Verification items for the finished model (mm, model axes). A direction names the side the tool comes from. Coordinates: 2 decimals unless noted, no trailing zeros. Write each loop counter-clockwise with the first axis right and the second up, starting at its lowest first coordinate (ties: lowest second). Pieces come first, ordered by that corner, then holes. Notation, with made-up numbers: (25, 7) -> (38, 7) arc R23 cw to (38, 41) -> close; hole circle Ø10 at (26.25, 33.25). An arc over 180 degrees is marked (long way). Answer in a Markdown table with one row per item.
```python
from build123d import *

# Parameters (mm, degrees)
EXTRUDE_1_DEPTH         = 115
SKETCH_2_W              = 200
SKETCH_2_H              = 37
EXTRUDE_2_DEPTH         = 30
EXTRUDE_3_DEPTH         = 20
SKETCH_4_R              = 22.5
CUT_EXTRUDE_1_DEPTH     = 2
SKETCH_5_R              = 18.5
CUT_EXTRUDE_2_DEPTH     = 8
CUT_EXTRUDE_3_REACH     = 169.29
SKETCH_6_R              = 23.5
SKETCH_7_R              = 9.5
CUT_EXTRUDE_4_DEPTH     = 85
SKETCH_8_R              = 6.5
CUT_EXTRUDE_5_DEPTH     = 154.186161255
SKETCH_9_R              = 2.5
CUT_EXTRUDE_6_DEPTH     = 10
FILLET_1_R              = 5
SKETCH_10_R             = 1
CUT_EXTRUDE_7_DEPTH     = 5
M5X0_8_1_D              = 4.2
M5X0_8_1_DEPTH          = 11
M5X0_8_1_TIP            = 1.2618073
HOLE_WIZARD_M10_1_D     = 8.5
HOLE_WIZARD_M10_1_DEPTH = 24
HOLE_WIZARD_M10_1_TIP   = 2.553657631
SKETCH_15_R             = 6.5
CUT_EXTRUDE_8_DEPTH     = 55
SKETCH_16_R             = 9.5
CUT_EXTRUDE_9_DEPTH     = 12


with BuildPart() as part:
    # 草图1 → 拉伸1 (new body)
    with BuildSketch(Plane.XY):
        Polygon((80, 0), (-80, 0), (-100, -20), (-100, -42), (100, -42), (100, -20), align=None)
    extrude(amount=EXTRUDE_1_DEPTH)

    # 草图2 → 拉伸2 (add)
    with BuildSketch(Plane.XY):
        with Locations((0, -60.5)):
            Rectangle(SKETCH_2_W, SKETCH_2_H)
    extrude(amount=EXTRUDE_2_DEPTH)

    # 草图3 → 拉伸3 (add)
    with BuildSketch(Plane.ZY.offset(100)):
        Polygon((115, -42), (30, -79), (30, -42), align=None)
    extrude_3 = extrude(amount=-EXTRUDE_3_DEPTH)

    # 镜向1: 拉伸3 across plane
    add(extrude_3.mirror(Plane(origin=(0, 0, 0), x_dir=(0, 0, 1), z_dir=(1, 0, 0))))

    # 草图4 → 切除-拉伸1 (cut)
    with BuildSketch(Plane(origin=(0, 0, 0), x_dir=(1, 0, 0), z_dir=(0, 1, 0))):
        with Locations(Location((0, -70, 0), (0, 0, 270))):
            Circle(SKETCH_4_R)
    extrude(amount=-CUT_EXTRUDE_1_DEPTH, mode=Mode.SUBTRACT)

    # 草图5 → 切除-拉伸2 (cut)
    with BuildSketch(Plane(origin=(0, -2, 0), x_dir=(1, 0, 0), z_dir=(0, 1, 0))):
        with Locations(Location((0, -70, 0), (0, 0, 270))):
            Circle(SKETCH_5_R)
    extrude(amount=-CUT_EXTRUDE_2_DEPTH, mode=Mode.SUBTRACT)

    # 草图6 → 切除-拉伸3 (cut, up to next)
    with BuildSketch(Plane(origin=(0, -10, 0), x_dir=(1, 0, 0), z_dir=(0, 1, 0)), mode=Mode.PRIVATE) as cut_extrude_3_sk1:
        with Locations(Location((0, -70, 0), (0, 0, 270))):
            Circle(SKETCH_6_R)
    cut_extrude_3_tool1 = extrude(cut_extrude_3_sk1.sketch, amount=-CUT_EXTRUDE_3_REACH, mode=Mode.PRIVATE) & part.part
    add(cut_extrude_3_tool1.solids().sort_by_distance((0, -10, 70))[0], mode=Mode.SUBTRACT)

    # 草图7 → 切除-拉伸4 (cut)
    with BuildSketch(Plane.XY.offset(115)):
        with Locations((60, -21)):
            Circle(SKETCH_7_R)
        with Locations((-60, -21)):
            Circle(SKETCH_7_R)
    extrude(amount=-CUT_EXTRUDE_4_DEPTH, mode=Mode.SUBTRACT)

    # 草图8 → 切除-拉伸5 (cut, through all)
    with BuildSketch(Plane.XY.offset(30)):
        with Locations((-60, -21)):
            Circle(SKETCH_8_R)
        with Locations((60, -21)):
            Circle(SKETCH_8_R)
    extrude(amount=-CUT_EXTRUDE_5_DEPTH, mode=Mode.SUBTRACT)

    # 草图9 → 切除-拉伸6 (cut)
    with BuildSketch(Plane.XZ.offset(42)):
        with Locations(Location((0, 104, 0), (0, 0, 270))):
            Circle(SKETCH_9_R)
        with Locations(Location((29.444863729, 87, 0), (0, 0, 270))):
            Circle(SKETCH_9_R)
        with Locations(Location((29.444863729, 53, 0), (0, 0, 270))):
            Circle(SKETCH_9_R)
        with Locations(Location((-29.444863729, 87, 0), (0, 0, 270))):
            Circle(SKETCH_9_R)
        with Locations(Location((-29.444863729, 53, 0), (0, 0, 270))):
            Circle(SKETCH_9_R)
    extrude(amount=-CUT_EXTRUDE_6_DEPTH, mode=Mode.SUBTRACT)

    # 圆角1
    fillet_1_edges = [part.edges().sort_by_distance(p)[0] for p in [
        (-80, -60.5, 30),
        (-80, -42, 72.5),
        (0, -42, 30),
        (80, -42, 72.5),
        (80, -60.5, 30),
    ]]
    fillet(fillet_1_edges, radius=FILLET_1_R)

    # 草图10 → 切除-拉伸7 (cut)
    with BuildSketch(Plane(origin=(0, 0, 0), x_dir=(1, 0, 0), z_dir=(0, 1, 0))):
        with Locations(Location((0, -38, 0), (0, 0, 270))):
            Circle(SKETCH_10_R)
        with Locations(Location((32, -70, 0), (0, 0, 270))):
            Circle(SKETCH_10_R)
        with Locations(Location((0, -102, 0), (0, 0, 270))):
            Circle(SKETCH_10_R)
        with Locations(Location((-32, -70, 0), (0, 0, 270))):
            Circle(SKETCH_10_R)
    extrude(amount=-CUT_EXTRUDE_7_DEPTH, mode=Mode.SUBTRACT)

    # M5x0.8 螺纹孔1
    with Locations(Plane(origin=(0, 0, 0), x_dir=(-1, 0, 0), z_dir=(0, 1, 0))):
        with Locations((0, 38), (-32, 70), (0, 102), (32, 70)):
            Hole(M5X0_8_1_D / 2, depth=M5X0_8_1_DEPTH)
            with Locations((0, 0, -(M5X0_8_1_DEPTH + M5X0_8_1_TIP / 2))):  # 118° drill point
                Cone(0, M5X0_8_1_D / 2, M5X0_8_1_TIP, mode=Mode.SUBTRACT)

    # M10 螺纹孔1
    with Locations(Plane.XZ.offset(42)):
        with Locations((29.444863729, 53), (29.444863729, 87), (0, 104), (-29.444863729, 87), (-29.444863729, 53)):
            Hole(HOLE_WIZARD_M10_1_D / 2, depth=HOLE_WIZARD_M10_1_DEPTH)
            with Locations((0, 0, -(HOLE_WIZARD_M10_1_DEPTH + HOLE_WIZARD_M10_1_TIP / 2))):  # 118° drill point
                Cone(0, HOLE_WIZARD_M10_1_D / 2, HOLE_WIZARD_M10_1_TIP, mode=Mode.SUBTRACT)

    # 草图15 → 切除-拉伸8 (cut)
    with BuildSketch(Plane.XY.offset(30)):
        with Locations((-60, -65)):
            Circle(SKETCH_15_R)
        with Locations((60, -65)):
            Circle(SKETCH_15_R)
    extrude(amount=-CUT_EXTRUDE_8_DEPTH, mode=Mode.SUBTRACT)

    # 草图16 → 切除-拉伸9 (cut)
    with BuildSketch(Plane.XY.offset(30)):
        with Locations((-60, -65)):
            Circle(SKETCH_16_R)
        with Locations((60, -65)):
            Circle(SKETCH_16_R)
    extrude(amount=-CUT_EXTRUDE_9_DEPTH, mode=Mode.SUBTRACT)


solid = part.part
```
1. Access from +Z, -Z, +X, -X, +Y, -Y to the whole of each face (thin tool, end or side, straight path). Record for faces 5 (the face through (1, 0, 44)), 6 (the face through (27.48, -29.83, 83.23)), 7 (the face through (32.08, -12.04, 69.64)), 8 (the face through (-78, -43, 76)), 9 (the face through (69.061, -18.146, 73.095)).
Findings below:
| item | result |
|---|---|
| face 5 | +Z, -Z, +X, -X, +Y |
| face 6 | -Y |
| face 7 | +Y |
| face 8 | +Z, -Y |
| face 9 | +Z |
2. Release check for a two-part mould opening along Y. For faces 1 (the face through (-51.224, -68.639, 24.084)), 2 (the face through (-18, -2, 65)), 3 (the face through (-78, -63, 31)), 4 (the face through (1, -43, 32)) record: released by +Y, released by -Y, zero draft, split by the parting line, or undercut.
Findings below:
| item | result |
|---|---|
| face 1 | undercut |
| face 2 | released by +Y |
| face 3 | zero draft |
| face 4 | released by -Y |
3. Material ranges on probe 1 along Y at (x, z) = (60, 20.5); probe 2 along Z at (x, y) = (32, -4); probe 3 along Y at (x, z) = (-60, 15), recorded low to high. Write a range as from..to.
Findings below:
| item | result |
|---|---|
| probe 1 | y = -79..-74.5, -55.5..-27.5, -14.5..0 |
| probe 2 | z = 0..67.9, 72.1..115 |
| probe 3 | y = -79..-71.5, -58.5..-27.5, -14.5..0 |
4. Sectioned sample at A-A, the plane y = -68. Record the cut outline in (x, z), and give its area (3 significant figures).
Findings below:
| item | result |
|---|---|
| outline | (-100, 0) -> (-65.77, 0) -> (-65.77, 18) -> (-69.01, 18) -> (-69.01, 30) -> (-75, 30) arc R5 cw to (-80, 35) -> (-80, 55.27) -> (-100, 55.27) -> close; (-54.23, 0) -> (54.23, 0) -> (54.23, 18) -> (50.99, 18) -> (50.99, 30) -> (-50.99, 30) -> (-50.99, 18) -> (-54.23, 18) -> close; (65.77, 0) -> (100, 0) -> (100, 55.27) -> (80, 55.27) -> (80, 35) arc R5 cw to (75, 30) -> (69.01, 30) -> (69.01, 18) -> (65.77, 18) -> close |
| area | 6,170 mm² |
5. Sectioned sample at B-B, the plane x = -61. Record the cut outline in (y, z).
Findings below:
| item | result |
|---|---|
| outline | (-79, 0) -> (-71.42, 0) -> (-71.42, 18) -> (-74.45, 18) -> (-74.45, 30) -> (-79, 30) -> close; (-58.58, 0) -> (-27.42, 0) -> (-27.42, 30) -> (-30.45, 30) -> (-30.45, 115) -> (-42, 115) -> (-42, 35) arc R5 cw to (-47, 30) -> (-55.55, 30) -> (-55.55, 18) -> (-58.58, 18) -> close; (-14.58, 0) -> (0, 0) -> (0, 115) -> (-11.55, 115) -> (-11.55, 30) -> (-14.58, 30) -> close |
6. Go/stop test with flat-tipped pins: pin 1 (21 mm diameter, centred on x = 64.5, y = -66, fed in from +Z); pin 2 (10 mm diameter, centred on x = 29.44, z = 53, fed in from -Y); pin 3 (4 mm diameter, centred on x = 0, z = 102, fed in from +Y); pin 4 (11.5 mm diameter, centred on x = -60, y = -21, fed in from +Z). Record where each tip stops, or that it passes through.
Findings below:
| item | result |
|---|---|
| pin 1 | stops at z = 30 |
| pin 2 | stops at y = -42 |
| pin 3 | stops at y = -11.06 |
| pin 4 | passes through |
